Part model, mm, in its own coordinate system. A direction names the side the tool comes from. Coordinates: 2 decimals unless noted, no trailing zeros. Write each loop counter-clockwise with the first axis right and the second up, starting at its lowest first coordinate (ties: lowest second). Pieces come first, ordered by that corner, then holes. Notation, with made-up numbers: (45, 24.25) - (103, 24.25) arc R35 ccw to (103, 58.25) - close; hole circle Ø11 at (-10.75, 72). An arc over 180 degrees is marked (long way). Use a Markdown table: item, result.
```python
from build123d import *

# Parameters (mm, degrees)
BASE_PLATE_SKETCH_W    = 85
BASE_PLATE_SKETCH_H    = 100
BASE_PLATE_DEPTH       = 15
UPRIGHT_WALL_DEPTH     = 15
SIDE_WALL_SKETCH_W     = 50
SIDE_WALL_SKETCH_H     = 65
SIDE_WALL_DEPTH        = 15
GUSSET_DEPTH           = 15
POST_SKETCH_W          = 20
POST_SKETCH_H          = 15
POST_DEPTH             = 60
STEPPED_BLOCK_DEPTH    = 15
MOUNTING_HOLE_SKETCH_R = 11.636423048
MOUNTING_HOLE_DEPTH    = 15


with BuildPart() as part:
    # Base Plate Sketch → Base Plate (new body)
    with BuildSketch(Plane(origin=(0, 0, 0), x_dir=(1, 0, 0), z_dir=(0, 1, 0))):
        Rectangle(BASE_PLATE_SKETCH_W, BASE_PLATE_SKETCH_H)
    extrude(amount=BASE_PLATE_DEPTH)

    # Upright Wall Sketch → Upright Wall (add)
    with BuildSketch(Plane(origin=(42.5, 0, 0), x_dir=(0, 0, -1), z_dir=(1, 0, 0))):
        Polygon((0, 15), (50, 15), (50, 80), (35, 80), (35, 60), (0, 60), align=None)
    extrude(amount=-UPRIGHT_WALL_DEPTH)

    # Side Wall Sketch → Side Wall (add)
    with BuildSketch(Plane.ZY.offset(42.5)):
        with Locations((-25, 47.5)):
            Rectangle(SIDE_WALL_SKETCH_W, SIDE_WALL_SKETCH_H)
    extrude(amount=-SIDE_WALL_DEPTH)

    # Gusset Sketch → Gusset (add)
    with BuildSketch(Plane.ZY.offset(42.5)):
        Polygon((0, 80), (50, 15), (0, 15), align=None)
    extrude(amount=-GUSSET_DEPTH)

    # Post Sketch → Post (add)
    with BuildSketch(Plane(origin=(0, 80, 0), x_dir=(1, 0, 0), z_dir=(0, 1, 0))):
        with Locations((-17.5, 7.5)):
            Rectangle(POST_SKETCH_W, POST_SKETCH_H)
    extrude(amount=-POST_DEPTH)

    # Stepped Block Sketch → Stepped Block (add)
    with BuildSketch(Plane.XY):
        Polygon((12.5, 40), (12.5, 60), (27.5, 60), (27.5, 15), (-7.5, 15), (-27.5, 14.790865335), (-27.5, 40), (-7.5, 40), align=None)
    extrude(amount=-STEPPED_BLOCK_DEPTH)

    # Mounting Hole Sketch → Mounting Hole (cut)
    with BuildSketch(Plane(origin=(0, 15, 0), x_dir=(1, 0, 0), z_dir=(0, 1, 0))):
        with Locations(Location((7.5, -25, 0), (0, 0, 270))):
            Circle(MOUNTING_HOLE_SKETCH_R)
    extrude(amount=-MOUNTING_HOLE_DEPTH, mode=Mode.SUBTRACT)


solid = part.part
```
Item 1: Which spindle directions (+Z, -Z, +X, -X, +Y, -Y) get a long thin tool onto all of the face, cutting with end or side? Do faces 4 (the face through (0, 15, -33)), 5 (the face through (-7.5, 60, -7)), 6 (the face through (-1, 15, 14)). Say none if no direction does.
From the geometry:
| item | result |
|---|---|
| face 4 | -Z, +Y |
| face 5 | +Z, -Z, +Y |
| face 6 | +Z, +X, +Y |
Item 2: Band-saw the part on C-C, the plane y = 71.5. Give the cut face in (x, z), then the cut area to 3 significant figures.
From the geometry:
| item | result |
|---|---|
| outline | (-42.5, -50) - (-27.5, -50) - (-27.5, -15) - (-7.5, -15) - (-7.5, 0) - (-27.5, 0) - (-27.5, 6.54) - (-42.5, 6.54) - close; (27.5, -50) - (42.5, -50) - (42.5, -35) - (27.5, -35) - close |
| area | 1,370 mm^2 |
Item 3: Band-saw the part on D-D, the plane x = -23.5. Give the cut face in (y, z), then the cut area to 4 significant figures.
From the geometry:
| item | result |
|---|---|
| outline | (0, -50) - (15, -50) - (15, -15) - (80, -15) - (80, 0) - (15, 0) - (15, 50) - (0, 50) - close |
| area | 2,475 mm^2 |
Item 4: Band-saw the part on A-A, the plane x = 7.5. Give the cut face in (y, z).
From the geometry:
| item | result |
|---|---|
| outline | (0, -50) - (15, -50) - (15, -15) - (40, -15) - (40, 0) - (15, 0) - (15, 13.36) - (0, 13.36) - close; (0, 36.64) - (15, 36.64) - (15, 50) - (0, 50) - close |
Item 5: Drop flat-ended pins along their axis: P1, Ø5, axis at x = 23.5, y = 41.5, coming from the -Z side; P2, Ø7.5, axis at x = 38, y = 71, coming from the +Z side; P3, Ø12, axis at y = 70, z = -10, coming from the +X side. Give the stop position or say it passes through.
From the geometry:
| item | result |
|---|---|
| P1 | z = -15 |
| P2 | z = -35 |
| P3 | x = -7.5 |
Item 6: Two-plate mould, pull along X, no slides. Class faces 1 (the face through (31, 60, -13)), 2 (the face through (42.5, 32, -10)), 3 (the face through (3, 40, -7)): pulls with the +X half, pulls with the -X half, needs draft (parallel to the pull), parting line crosses it, or undercut.
From the geometry:
| item | result |
|---|---|
| face 1 | needs draft |
| face 2 | pulls with the +X half |
| face 3 | undercut |
Item 7: Drill centre lines: probe 1 along X at (y, z) = (46.5, -13.5); probe 2 along X at (y, z) = (8, 25.5); probe 3 along Y at (x, z) = (-19, 8). Where is each one in solid material? Low to high.
From the geometry:
| item | result |
|---|---|
| probe 1 | -42.5 to -7.5, 12.5 to 42.5 |
| probe 2 | -42.5 to -4.13, 19.13 to 42.5 |
| probe 3 | 0 to 15 |
Item 8: Band-saw the part on B-B, the plane z = 25. Give the cut face in (x, y).
From the geometry:
| item | result |
|---|---|
| outline | (-42.5, 0) - (-4.14, 0) - (-4.14, 15) - (-27.5, 15) - (-27.5, 47.5) - (-42.5, 47.5) - close; (19.14, 0) - (42.5, 0) - (42.5, 15) - (19.14, 15) - close |
